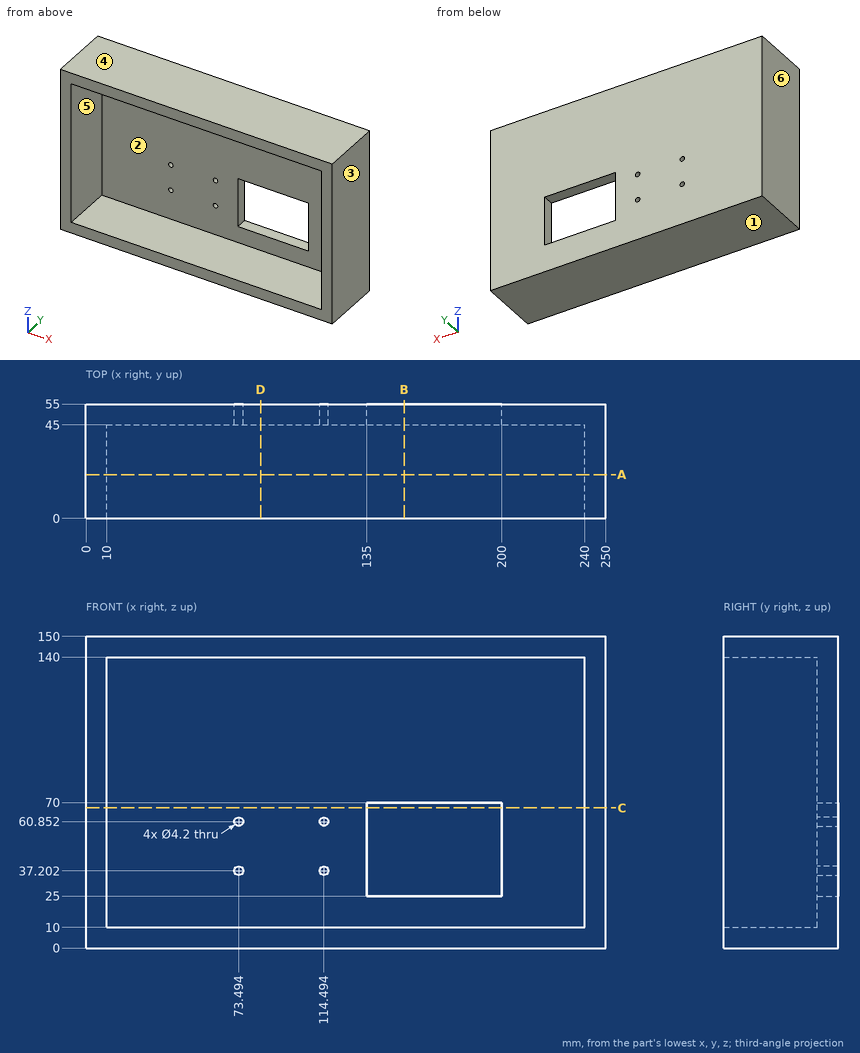
Can you work these out from the drawing? Everything is in mm from the part's minimum corner. A direction names the side the tool comes from. Round coordinates to 2 decimals unless told otherwise and drop trailing zeros. Loops run counter-clockwise (first coordinate to the right, second up) from the corner with the lowest first, then second, coordinate; pieces in that order, holes last. Notation, with made-up numbers: (0.25, 41.25) - (59.25, 41.25) arc R17 ccw to (59.25, 70.25) - close; hole circle Ø4 at (42.5, 19). An arc over 180 degrees is marked (long way). Answer in a Markdown table with one row per item. Add a question column.
(1) If we section it at C-C (z = 67.5): Please give me the cut outline in (x, y), plus the area to 3 significant figures.
(2) I'm going to push a flat-ended pin straight in: pin 1 (5.5 mm diameter, centred on x = 73.49, z = 60.85, fed in from -Y). Where does the tip first touch, or does it pass through?
(3) If we section it at B-B (x = 153): Please give me the cut outline in (y, z).
(4) If we section it at D-D (x = 84): Please give me the cut outline in (y, z).
(5) I need wall thicknesses on line 1 along Z through (x, y) = (231, 28); line 2 along X through (y, z) = (3, 52); line 3 along Z through (x, y) = (137, 52.5). Which ranges of each line are inside material? Lowest first, please.
(6) If we mould it in two halves opening along Z, with no side actions, what happens to the marked faces 1, 2, 3 and 4? For each: pulls with the +Z half, pulls with the -Z half, needs draft (parallel to the pull), parting line crosses it, or undercut.
(7) If we section it at A-A (y = 21): Please give me the cut outline in (x, z), plus the area to 3 significant figures.
(8) For the marked faces 5 and 6, which set-ups out of +Z, -Z, +X, -X, +Y, -Y let a thin tool reach every point of the face, with its end or its side?
Model answer:
| question | item | result |
|---|---|---|
| 1 | outline | (0, 0) - (10, 0) - (10, 45) - (135, 45) - (135, 55) - (0, 55) - close; (200, 45) - (240, 45) - (240, 0) - (250, 0) - (250, 55) - (200, 55) - close |
| 1 | area | 2,750 mm² |
| 2 | pin 1 | stops at y = 45 |
| 3 | outline | (0, 0) - (55, 0) - (55, 25) - (45, 25) - (45, 10) - (0, 10) - close; (0, 140) - (45, 140) - (45, 70) - (55, 70) - (55, 150) - (0, 150) - close |
| 4 | outline | (0, 0) - (55, 0) - (55, 150) - (0, 150) - (0, 140) - (45, 140) - (45, 10) - (0, 10) - close |
| 5 | line 1 | z = 0 to 10, 140 to 150 |
| 5 | line 2 | x = 0 to 10, 240 to 250 |
| 5 | line 3 | z = 0 to 25, 70 to 150 |
| 6 | face 1 | pulls with the -Z half |
| 6 | face 2 | undercut |
| 6 | face 3 | needs draft |
| 6 | face 4 | pulls with the +Z half |
| 7 | outline | (0, 0) - (250, 0) - (250, 150) - (0, 150) - close; hole (10, 10) - (240, 10) - (240, 140) - (10, 140) - close |
| 7 | area | 7,600 mm² |
| 8 | face 5 | -Y |
| 8 | face 6 | +Z, -Z, -X, +Y, -Y |
